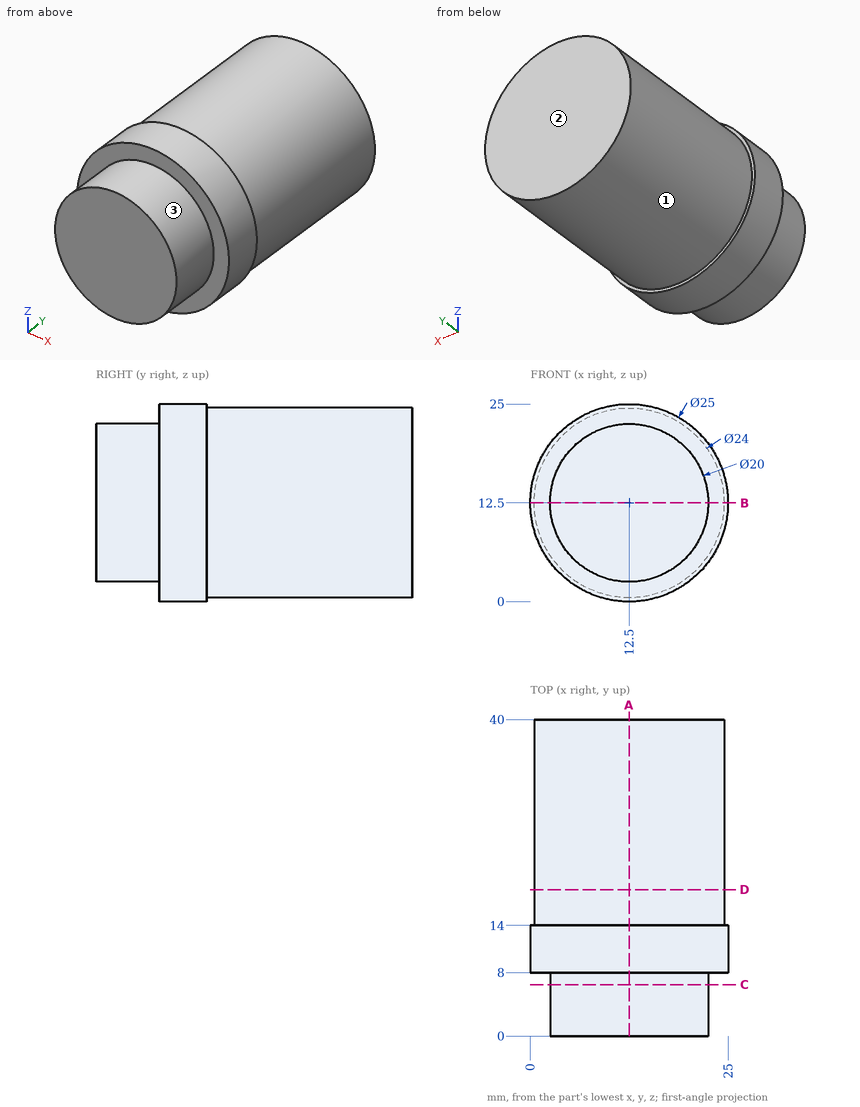
Answer from the drawing. Dimensions are ordinates in mm from the lowest x, y and z of the part. A direction names the side the tool comes from. Give positions to 0.01 mm unless a question says otherwise; leave off trailing zeros. Loops run counter-clockwise (first coordinate to the right, second up) from the corner with the lowest first, then second, coordinate; pieces in that order, holes last. Notation, with made-up numbers: (13.5, -11.75) -> (53.5, -11.75) arc R16 cw to (53.5, 17.25) -> close; hole circle Ø3 at (31, 80). An arc over 180 degrees is marked (long way). Answer as CSV lines item,"result".
Item 1: Find section B-B on z = 12.5. Give the vertices of the cut face in (x, y), plus the area to 3 significant figures.
Returned:
outline,"(0, 8) -> (2.5, 8) -> (2.5, 0) -> (22.5, 0) -> (22.5, 8) -> (25, 8) -> (25, 14) -> (24.5, 14) -> (24.5, 40) -> (0.5, 40) -> (0.5, 14) -> (0, 14) -> close"
area,"934 mm²"
Item 2: Each of these flat-tipped pins is pushed along its axis until it touches: pin 1 (2 mm diameter, centred on y = 25.5, z = 22, fed in from +X); pin 2 (2 mm diameter, centred on y = 26, z = 4, fed in from -X); pin 3 (1.5 mm diameter, centred on y = 25.5, z = 17.5, fed in from +X). Where does it stop, or does it pass through?
Returned:
pin 1,"stops at x = 20.97"
pin 2,"stops at x = 3.13"
pin 3,"stops at x = 23.72"
Item 3: For the marked faces 1, 2 and 3, determine the directions among +Z, -Z, +X, -X, +Y, -Y from which every point of the face is accessible in a straight line to the end or side of a thin tool.
Returned:
face 1,"+Y"
face 2,"+Z, -Z, +X, -X, +Y"
face 3,"-Y"
Item 4: Find section D-D on y = 18.5. Give the vertices of the cut face in (x, z), plus the area to 3 significant figures.
Returned:
outline,"circle Ø24 at (12.5, 12.5)"
area,"452 mm²"
Item 5: Find section A-A on x = 12.5. Give the vertices of the cut face in (y, z), plus the area to 3 significant figures.
Returned:
outline,"(0, 2.5) -> (8, 2.5) -> (8, 0) -> (14, 0) -> (14, 0.5) -> (40, 0.5) -> (40, 24.5) -> (14, 24.5) -> (14, 25) -> (8, 25) -> (8, 22.5) -> (0, 22.5) -> close"
area,"934 mm²"
Item 6: Consider line 1 (X direction, y = 2, z = 12.75); line 2 (X direction, y = 19.5, z = 12); line 3 (Y direction, x = 4, z = 6). Determine where each line is inside the solid, lowest interval first. Write a range as [from, to].
Returned:
line 1,"x = [2.5, 22.5]"
line 2,"x = [0.51, 24.49]"
line 3,"y = [8, 40]"
Item 7: Find section C-C on y = 6.5. Give the vertices of the cut face in (x, z), plus the area to 3 significant figures.
Returned:
outline,"circle Ø20 at (12.5, 12.5)"
area,"314 mm²"
